```python
from build123d import *

# Parameters (mm, degrees)
BOSS_EXTRUDE1_DEPTH     = 2
CUT_EXTRUDE1_DEPTH      = 42.707695968
CUT_EXTRUDE1_DEPTH_BACK = 42.707695968
SKETCH3_R               = 1.5
SKETCH3_R_2             = 1.472115529
SKETCH3_R_3             = 1.512476654
CUT_EXTRUDE2_DEPTH      = 42.707695968
SKETCH4_R               = 2
CUT_EXTRUDE3_DEPTH      = 42.707695968


with BuildPart() as part:
    # Sketch1 → Boss-Extrude1 (new body)
    with BuildSketch(Plane.XY):
        with BuildLine():
            Line((-22.843450479, 26.485623003), (27.156549521, 26.485623003))
            ThreePointArc((27.156549521, 26.485623003), (30.692083427, 25.021156909), (32.156549521, 21.485623003))
            Line((32.156549521, 21.485623003), (32.156549521, -8.514376997))
            ThreePointArc((32.156549521, -8.514376997), (30.692083427, -12.049910903), (27.156549521, -13.514376997))
            Line((27.156549521, -13.514376997), (-22.843450479, -13.514376997))
            ThreePointArc((-22.843450479, -13.514376997), (-26.378984385, -12.049910903), (-27.843450479, -8.514376997))
            Line((-27.843450479, -8.514376997), (-27.843450479, 21.485623003))
            ThreePointArc((-27.843450479, 21.485623003), (-26.378984385, 25.021156909), (-22.843450479, 26.485623003))
        make_face()
    extrude(amount=BOSS_EXTRUDE1_DEPTH)

    # Sketch2 → Cut-Extrude1 (cut, two sides: drawn at the far end of the back side and taken through both)
    with BuildSketch(Plane.XY.offset(2).offset(-CUT_EXTRUDE1_DEPTH_BACK)):
        with BuildLine():
            Line((-17.075923419, 11.875959063), (21.38902246, 11.875959063))
            ThreePointArc((21.38902246, 11.875959063), (22.096129242, 11.583065844), (22.38902246, 10.875959063))
            Line((22.38902246, 10.875959063), (22.38902246, -7.624040937))
            ThreePointArc((22.38902246, -7.624040937), (22.096129242, -8.331147718), (21.38902246, -8.624040937))
            Line((21.38902246, -8.624040937), (-17.075923419, -8.624040937))
            ThreePointArc((-17.075923419, -8.624040937), (-17.7830302, -8.331147718), (-18.075923419, -7.624040937))
            Line((-18.075923419, -7.624040937), (-18.075923419, 10.875959063))
            ThreePointArc((-18.075923419, 10.875959063), (-17.7830302, 11.583065844), (-17.075923419, 11.875959063))
        make_face()
    extrude(amount=CUT_EXTRUDE1_DEPTH + CUT_EXTRUDE1_DEPTH_BACK, mode=Mode.SUBTRACT)

    # Sketch3 → Cut-Extrude2 (cut, through all)
    with BuildSketch(Plane.XY.offset(2)):
        with Locations((2.156549521, 15.875959063)):
            Circle(SKETCH3_R)
        with Locations((12.156549521, 21.525959063)):
            Circle(SKETCH3_R_2)
        with Locations((-7.843450479, 21.525959063)):
            Circle(SKETCH3_R_3)
    extrude(amount=-CUT_EXTRUDE2_DEPTH, mode=Mode.SUBTRACT)

    # Sketch4 → Cut-Extrude3 (cut, through all)
    with BuildSketch(Plane.XY.offset(2)):
        with Locations((27.17171292, -3.424040937)):
            Circle(SKETCH4_R)
        with Locations((27.17171292, 6.575959063)):
            Circle(SKETCH4_R)
        with Locations(Location((-22.858613878, -3.424040937, 0), (0, 0, 180))):
            Circle(SKETCH4_R)
        with Locations(Location((-22.858613878, 6.575959063, 0), (0, 0, 180))):
            Circle(SKETCH4_R)
    extrude(amount=-CUT_EXTRUDE3_DEPTH, mode=Mode.SUBTRACT)


solid = part.part
```
Model file for the job. Use its own axes, mm. A direction names the side the tool comes from. Round coordinates to 2 decimals unless told otherwise and drop trailing zeros. Order: outer loops, then holes, each group sorted by start corner. A loop starts at its lowest first (then second) coordinate and runs counter-clockwise, first axis right, second up. Notation, with made-up numbers: (88.25, 33.5) -> (129.25, 33.5) arc R16 cw to (129.25, 40.5) -> close; hole circle Ø11 at (-39.75, 85.5). An arc over 180 degrees is marked (long way). Use one line per item in the form item = value.
Item 1: Cut at C-C, the plane x = -8.5. Write the cut outline in (y, z), and give its area (3 significant figures).
Returned:
outline = (-13.51, 0) -> (-8.62, 0) -> (-8.62, 2) -> (-13.51, 2) -> close; (11.88, 0) -> (20.16, 0) -> (20.16, 2) -> (11.88, 2) -> close; (22.89, 0) -> (26.49, 0) -> (26.49, 2) -> (22.89, 2) -> close
area = 33.5 mm^2
Item 2: Cut at A-A, the plane y = 1.5. Write the cut outline in (x, z), and give its area (3 significant figures).
Returned:
outline = (-27.84, 0) -> (-18.08, 0) -> (-18.08, 2) -> (-27.84, 2) -> close; (22.39, 0) -> (32.16, 0) -> (32.16, 2) -> (22.39, 2) -> close
area = 39.1 mm^2
Item 3: Drill centre lines: line 1 (Y direction, x = 20, z = 1.85); line 2 (X direction, y = 0, z = 0.7); line 3 (Y direction, x = 2, z = 0.95). Where is each one in solid material? Low to high.
Returned:
line_1 = -13.51 to -8.62, 11.88 to 26.49
line_2 = -27.84 to -18.08, 22.39 to 32.16
line_3 = -13.51 to -8.62, 11.88 to 14.38, 17.37 to 26.49
Item 4: Cut at B-B, the plane x = 9. Write the cut outline in (y, z), and give its area (3 significant figures).
Returned:
outline = (-13.51, 0) -> (-8.62, 0) -> (-8.62, 2) -> (-13.51, 2) -> close; (11.88, 0) -> (26.49, 0) -> (26.49, 2) -> (11.88, 2) -> close
area = 39.0 mm^2
Item 5: Tool access for faces 1 (the face through (-18.076, 1, 1)), 2 (the face through (-26.34, -12.09, 0.99)): list every direction of +Z, -Z, +X, -X, +Y, -Y with a clear straight run to the whole face (end or side of a thin tool).
Returned:
face_1 = +Z, -Z
face_2 = +Z, -Z, -X, -Y
Item 6: Cut at D-D, the plane z = 0.6. Give the number of separate pieces and of enclosed holes in the cut face, and give its area (3 significant figures).
Returned:
separate_pieces = 1
enclosed_holes = 8
area = 1,480 mm^2
Item 7: Pull direction X, two halves, no side cores. Call faces 3 (the face through (2, -8.624, 1)), 4 (the face through (-26.4, 25, 1)), 5 (the face through (9, 16, 2)), 6 (the face through (2, 11.876, 1)): released by +X, released by -X, zero draft, split by the parting line, or undercut.
Returned:
face_3 = undercut
face_4 = released by -X
face_5 = zero draft
face_6 = undercut
